from build123d import *

# Parameters (mm, degrees)
SKETCH1_W             = 354
SKETCH1_H             = 8
M6_TAPPED_HOLE1_D     = 5
M6_TAPPED_HOLE1_DEPTH = 15
M6_TAPPED_HOLE1_TIP   = 1.502151548
M6_TAPPED_HOLE2_D     = 5
M6_TAPPED_HOLE2_DEPTH = 15
M6_TAPPED_HOLE2_TIP   = 1.502151548


with BuildPart() as part:
    # Sketch1 → Revolve1 (revolve)
    with BuildSketch(Plane.XY, mode=Mode.PRIVATE) as revolve1_sk:
        with Locations((0, 4)):
            Rectangle(SKETCH1_W, SKETCH1_H)
    revolve(revolve1_sk.sketch.rotate(Axis((-177, 0, 0), (1, 0, 0)), 90), axis=Axis((-177, 0, 0), (1, 0, 0)))

    # M6 Tapped Hole1
    with Locations(Plane(origin=(177, 0, 0), x_dir=(0, 0, -1), z_dir=(1, 0, 0))):
        with Locations((0, 0)):
            Hole(M6_TAPPED_HOLE1_D / 2, depth=M6_TAPPED_HOLE1_DEPTH)
            with Locations((0, 0, -(M6_TAPPED_HOLE1_DEPTH + M6_TAPPED_HOLE1_TIP / 2))):  # 118° drill point
                Cone(0, M6_TAPPED_HOLE1_D / 2, M6_TAPPED_HOLE1_TIP, mode=Mode.SUBTRACT)

    # M6 Tapped Hole2
    with Locations(Plane.ZY.offset(177)):
        with Locations((0, 0)):
            Hole(M6_TAPPED_HOLE2_D / 2, depth=M6_TAPPED_HOLE2_DEPTH)
            with Locations((0, 0, -(M6_TAPPED_HOLE2_DEPTH + M6_TAPPED_HOLE2_TIP / 2))):  # 118° drill point
                Cone(0, M6_TAPPED_HOLE2_D / 2, M6_TAPPED_HOLE2_TIP, mode=Mode.SUBTRACT)


solid = part.part
Input: part model. Units: mm. Frame: model coordinates. Coordinates: 2 decimals unless noted, no trailing zeros. Write each loop counter-clockwise with the first axis right and the second up, starting at its lowest first coordinate (ties: lowest second). Pieces come first, ordered by that corner, then holes. Notation, with made-up numbers: M 72.5,-37 L 85.5,-37 A10 ccw 85.5,-22 Z; hole C 16,24.25 d5. An arc over 180 degrees is marked long. Answer as a JSON object with one key per item and string values. Group by question number.
(1) Section B-B on z = -5.25. Output: boundary loops of the cut face in (x, y), plus the area to 3 significant figures.
(2) Contact query for flat-ended pins moving along their axis: P1, Ø2, axis at x = 45, z = -3.5, coming from the +Y side; P2, Ø1.5, axis at x = -104, z = -3.5, coming from the -Y side. Output: stop coordinate, or through.
(3) Ray query, line 1 along Y through (x, z) = (171.5, 0); line 2 along Z through (x, y) = (35.5, 1.5); line 3 along Z through (x, y) = (30, -3.5). Return the intervals inside material, ascending. Write a range as [from, to].
(4) Section A-A on x = -80. Output: boundary loops of the cut face in (y, z).
Result set:
{
 "1": {"outline": "M -177,-6.04 L 177,-6.04 L 177,6.04 L -177,6.04 Z", "area": "4,270 mm2"},
 "2": {"P1": "stops at y = 7.6", "P2": "stops at y = -7.51"},
 "3": {"line 1": "y = [-8, -2.5], [2.5, 8]", "line 2": "z = [-7.86, 7.86]", "line 3": "z = [-7.19, 7.19]"},
 "4": {"outline": "C 0,0 d16"}
}
